from build123d import *

# Parameters (mm, degrees)
BOSS_EXTRUDE1_DEPTH = 8


with BuildPart() as part:
    # Sketch1 → Boss-Extrude1 (new body)
    with BuildSketch(Plane.XY):
        with BuildLine():
            Line((30, -25), (-30, -25))
            ThreePointArc((-30, -25), (-37.071067812, -22.071067812), (-40, -15))
            Line((-40, -15), (-40, 15))
            ThreePointArc((-40, 15), (-37.071067812, 22.071067812), (-30, 25))
            Line((-30, 25), (30, 25))
            ThreePointArc((30, 25), (37.071067812, 22.071067812), (40, 15))
            Line((40, 15), (40, -15))
            ThreePointArc((40, -15), (37.071067812, -22.071067812), (30, -25))
        make_face()
    extrude(amount=BOSS_EXTRUDE1_DEPTH)


solid = part.part
Source: CAD feature listing. Evaluate the final solid. Frame: model axes, mm. Round coordinates to 2 decimals unless told otherwise and drop trailing zeros. Loops run counter-clockwise (first coordinate to the right, second up) from the corner with the lowest first, then second, coordinate; pieces in that order, holes last.
Q1. Section A-A, the plane z = 3.75. Return loops of the section in (x, y), plus the area to 3 significant figures.
Q2. First-contact query: P1, Ø2, axis at x = 3, y = -10, coming from the -Z side. Flat tip, straight axial feed; report the tip coordinate or a pass-through.
Q3. Ray query, line 1 (X direction, y = -22, z = 6); line 2 (Y direction, x = -31, z = 0.5); line 3 (X direction, y = 17.5, z = 4.75). Return the intervals inside material, ascending.
Q4. Section B-B, the plane y = 21. Return loops of the section in (x, z), plus the area to 3 significant figures.
Solutions:
1. outline: (-40, -15) arc R10 ccw to (-30, -25) - (30, -25) arc R10 ccw to (40, -15) - (40, 15) arc R10 ccw to (30, 25) - (-30, 25) arc R10 ccw to (-40, 15) - close
1. area: 3,910 mm2
2. P1: stops at z = 0
3. line 1: x = -37.14 to 37.14
3. line 2: y = -24.95 to 24.95
3. line 3: x = -39.68 to 39.68
4. outline: (-38, 0) - (38, 0) - (38, 8) - (-38, 8) - close
4. area: 608 mm2
